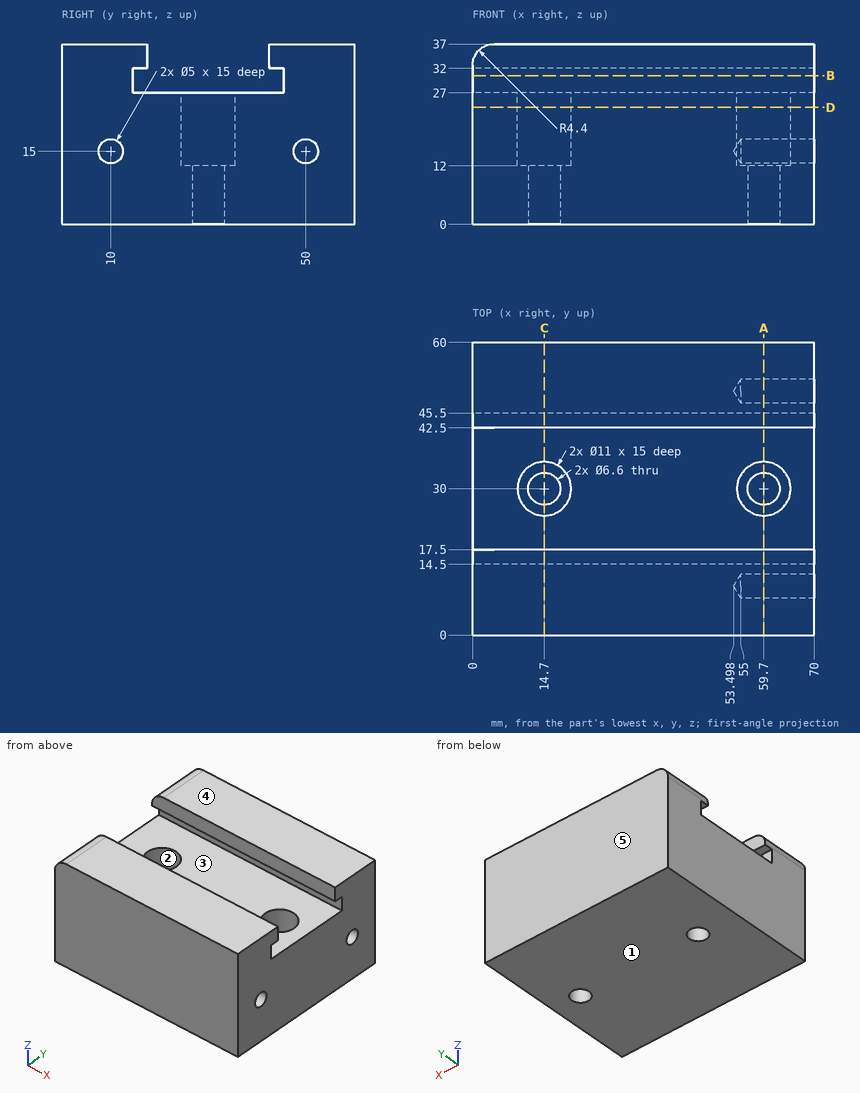
Input: dimensioned drawing with shaded views. Units: mm. Origin: part minimum x, y, z. A direction names the side the tool comes from. Coordinates: 2 decimals unless noted, no trailing zeros. Loops run counter-clockwise (first coordinate to the right, second up) from the corner with the lowest first, then second, coordinate; pieces in that order, holes last. Notation, with made-up numbers: (44, 0.5) - (75, 0.5) arc R37 cw to (75, 38.5) - close; hole circle Ø5 at (80.25, 70.5). An arc over 180 degrees is marked (long way). One line per question, with ' | ' between items. Start each with the question number.
(1) Reachability of the marked faces 1 and 2 from +Z, -Z, +X, -X, +Y, -Y: full face, straight path, thin tool, end or side. Return the list, or none.
(2) Cut plane B-B on z = 30.5. Output: boundary loops of the cut face in (x, y), and give its area (3 significant figures).
(3) Ray query, L1, parallel to Y at x = 59.7, z = 9.25; L2, parallel to Y at x = 60, z = 15; L3, parallel to Y at x = 59.7, z = 15.75 (1 decimal). Return the intervals inside material, ascending. Write a range as from..to.
(4) Draft query along Y for the marked faces 3, 4 and 5. Return one class per face: +Y half, -Y half, draft (parallel to the pull), parting line (faces both ways), or undercut.
(5) Cut plane A-A on x = 59.7. Output: boundary loops of the cut face in (y, z), and give its area (3 significant figures).
(6) First-contact query: pin 1 (12 mm diameter, centred on x = 61.5, y = 28.5, fed in from +Z); pin 2 (3.5 mm diameter, centred on x = 19, y = 44.5, fed in from -Z). Flat tips, straight axial feed; report the tip coordinate or a pass-through.
(7) Cut plane D-D on z = 24. Output: boundary loops of the cut face in (x, y), and give its area (3 significant figures).
(8) Cut plane C-C on x = 14.7. Output: boundary loops of the cut face in (y, z).
Here are the results:
1) face 1: -Z, +X, -X, +Y, -Y | face 2: +Z
2) outline: (0, 0) - (70, 0) - (70, 14.5) - (0, 14.5) - close; (0, 45.5) - (70, 45.5) - (70, 60) - (0, 60) - close | area: 2,030 mm²
3) L1: 0..26.7, 33.3..60 | L2: 0..7.5, 12.5..24.51, 35.49..47.5, 52.5..60 | L3: 0..7.6, 12.4..24.5, 35.5..47.6, 52.4..60
4) face 3: undercut | face 4: draft | face 5: +Y half
5) outline: (0, 0) - (26.7, 0) - (26.7, 12) - (24.5, 12) - (24.5, 27) - (14.5, 27) - (14.5, 32) - (17.5, 32) - (17.5, 37) - (0, 37) - close; (33.3, 0) - (60, 0) - (60, 37) - (42.5, 37) - (42.5, 32) - (45.5, 32) - (45.5, 27) - (35.5, 27) - (35.5, 12) - (33.3, 12) - close; hole circle Ø5 at (10, 15); hole circle Ø5 at (50, 15) | area: 1,660 mm²
6) pin 1: z = 27 | pin 2: z = 0
7) outline: (0, 0) - (70, 0) - (70, 60) - (0, 60) - close; hole circle Ø11 at (14.7, 30); hole circle Ø11 at (59.7, 30) | area: 4,010 mm²
8) outline: (0, 0) - (26.7, 0) - (26.7, 12) - (24.5, 12) - (24.5, 27) - (14.5, 27) - (14.5, 32) - (17.5, 32) - (17.5, 37) - (0, 37) - close; (33.3, 0) - (60, 0) - (60, 37) - (42.5, 37) - (42.5, 32) - (45.5, 32) - (45.5, 27) - (35.5, 27) - (35.5, 12) - (33.3, 12) - close
